```python
from build123d import *

# Parameters (mm, degrees)
SKETCH_1_R           = 16.5
BOSS_EXTRUDE_1_DEPTH = 13


with BuildPart() as part:
    # Sketch 1 → Boss-Extrude 1 (new, symmetric)
    with BuildSketch(Plane(origin=(0, 0, 0), x_dir=(1, 0, 0), z_dir=(0, 1, 0))):
        Polygon((0, 28.29016319), (-24.5, 14.145081595), (-24.5, -14.145081595), (0, -28.29016319), (24.5, -14.145081595), (24.5, 14.145081595), align=None)
        with Locations(Location((0, 0, 0), (0, 0, 90))):
            Circle(SKETCH_1_R, mode=Mode.SUBTRACT)
    extrude(amount=BOSS_EXTRUDE_1_DEPTH, both=True)

    # Sketch 2 → Cut-Revolve 1 (revolve, cut)
    with BuildSketch(Plane(origin=(0, 0, 0), x_dir=(0, 0, -1), z_dir=(1, 0, 0))):
        with BuildLine():
            Line((-22.29016319, 13), (-28.29016319, 13))
            Line((-28.29016319, 13), (-28.29016319, 10))
            add(Edge.make_bspline(
                [(-28.29016319, 10), (-27.028728561, 12.12896823), (-24.711520857, 13), (-22.29016319, 13)],
                knots=[0, 0, 0, 0, 1, 1, 1, 1], degree=3))
        make_face()
        with BuildLine():
            Line((-28.29016319, -13), (-28.29016319, -10))
            add(Edge.make_bspline(
                [(-28.29016319, -10), (-27.028728561, -12.12896823), (-24.711520857, -13), (-22.29016319, -13)],
                knots=[0, 0, 0, 0, 1, 1, 1, 1], degree=3))
            Line((-22.29016319, -13), (-28.29016319, -13))
        make_face()
    revolve(axis=Axis((0, 20.720193417, 0), (0, -1, 0)), mode=Mode.SUBTRACT)


solid = part.part
```
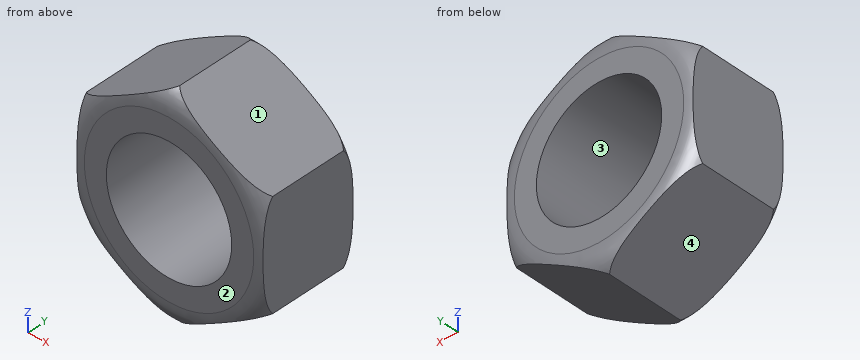
The model under review builds one solid part; all positions refer to its coordinate system, in mm. Face numbers are marked on the shaded views. Give positions to 0.01 mm unless a question says otherwise; leave off trailing zeros. Write each loop counter-clockwise with the first axis right and the second up, starting at its lowest first coordinate (ties: lowest second). Pieces come first, ordered by that corner, then holes. Notation, with made-up numbers: M -26,-40 L 30,-40 A19 ccw 30,-19 Z; hole C 50,61.25 d11. An arc over 180 degrees is marked long. Write each question's results on one line, items separated by ' | '. Start each with the question number.
1. We need section A-A (y = 6). Write out the cut boundary in (x, z).
2. Insertion check: pin 1 Ø6 at (y, z) = (2, -15.5) entering from +X; pin 2 Ø1 at (x, y) = (-15, -3.5) entering from +Z; pin 3 Ø2 at (y, z) = (10.5, 21.5) entering from -X. Each pin has a flat end and moves straight along its axis. Give the tip position at first contact, or say it passes through.
3. Mouldability with a two-part tool opening along Z and no side actions: class the marked faces 1, 2, 3 and 4 as released by +Z, released by -Z, zero draft, split by the parting line, or undercut.
4. For probe 1 along X at (y, z) = (-7, 0); probe 2 along Z at (x, y) = (-2, -9.75); probe 3 along Y at (x, z) = (-18, -13.5), list the stretches that pass through material, from the lowest coordinate up. Write a range as [from, to].
Results found:
1) outline: M -24.5,-14.15 L 0,-28.29 L 24.5,-14.15 L 24.5,14.15 L 0,28.29 L -24.5,14.15 Z; hole C 0,0 d33
2) pin 1: stops at x = 24.5 | pin 2: stops at z = 19.92 | pin 3: stops at x = -13.49
3) face 1: released by +Z | face 2: zero draft | face 3: undercut | face 4: released by -Z
4) probe 1: x = [-24.5, -16.5], [16.5, 24.5] | probe 2: z = [-27.14, -16.38], [16.38, 27.14] | probe 3: y = [-13, 13]
